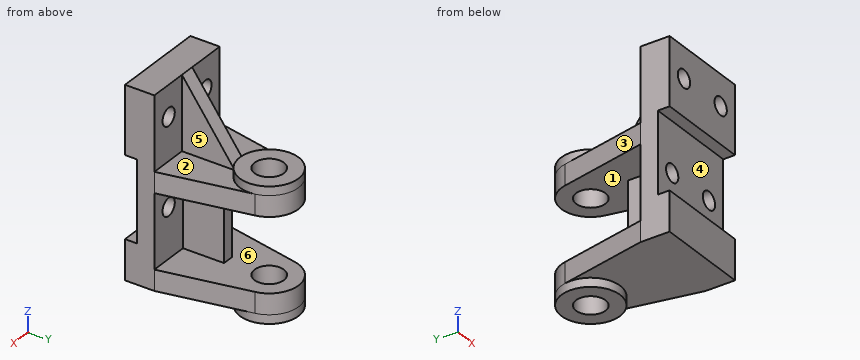
```python
from build123d import *

# Parameters (mm, degrees)
BASE_PLATE_DEPTH           = 32
LUG_UPRIGHT_PROFILE_R      = 10
LUG_UPRIGHT_DEPTH          = 14
LUG_START                  = 6
SKETCH2_3_R                = 20
SKETCH2_3_R_2              = 10
LUG_HUB_BOSS_DEPTH         = 6
BACK_WEB_PROFILE_W         = 8
BACK_WEB_PROFILE_H         = 50
BACK_WEB_DEPTH             = 28
STIFFENING_RIB_REACH       = 165.169
STIFFENING_RIB_PATH_WALL_W = 389.948936072
STIFFENING_RIB_PATH_WALL_H = 10
MOUNTING_HOLES_PROFILE_R   = 6
MOUNTING_HOLES_DEPTH       = 153.262930485


with BuildPart() as part:
    # Base Plate Profile → Base Plate (new, symmetric)
    with BuildSketch(Plane(origin=(0, 0, 0), x_dir=(0, 0, -1), z_dir=(1, 0, 0))):
        Polygon((-82, 0), (-128, 0), (-128, 20), (0, 20), (0, 0), (-27, 0), (-27, 8), (-82, 8), align=None)
    extrude(amount=BASE_PLATE_DEPTH, both=True)

    # Lug Upright Profile → Lug Upright (add)
    with BuildSketch(Plane(origin=(0, 0, 0), x_dir=(-1, 0, 0), z_dir=(0, 0, -1))):
        with BuildLine():
            Line((-19.585841233, 80.049052133), (-32, 20))
            Line((-32, 20), (32, 20))
            Line((32, 20), (19.585841233, 80.049052133))
            ThreePointArc((19.585841233, 80.049052133), (0, 96), (-19.585841233, 80.049052133))
        make_face()
        with Locations((0, 76)):
            Circle(LUG_UPRIGHT_PROFILE_R, mode=Mode.SUBTRACT)
    lug_upright = extrude(amount=-LUG_UPRIGHT_DEPTH)

    # Sketch2_3 → Lug Hub Boss (add)
    with BuildSketch(Plane(origin=(0, 0, 0), x_dir=(-1, 0, 0), z_dir=(0, 0, -1)).offset(LUG_START)):
        with Locations((0, 76)):
            Circle(SKETCH2_3_R)
        with Locations((0, 76)):
            Circle(SKETCH2_3_R_2, mode=Mode.SUBTRACT)
    lug_hub_boss = extrude(amount=-LUG_HUB_BOSS_DEPTH)

    # Lug Mirror: Lug Upright, Lug Hub Boss across plane
    add(lug_upright.mirror(Plane.XY.offset(39)))
    add(lug_hub_boss.mirror(Plane.XY.offset(39)))

    # Back Web Profile → Back Web (add)
    with BuildSketch(Plane(origin=(0, 20, 0), x_dir=(1, 0, 0), z_dir=(0, 1, 0))):
        with Locations((0, -39)):
            Rectangle(BACK_WEB_PROFILE_W, BACK_WEB_PROFILE_H)
    extrude(amount=BACK_WEB_DEPTH)

    # Stiffening Rib Path wall → Stiffening Rib (add, up to next)
    with BuildSketch(Plane(origin=(0, 38, 103), x_dir=(0, 0.584304725845, -0.811534341451), z_dir=(0, 0.811534341451, 0.584304725845)), mode=Mode.PRIVATE) as stiffening_rib_sk1:
        Rectangle(STIFFENING_RIB_PATH_WALL_W, STIFFENING_RIB_PATH_WALL_H)
    stiffening_rib_tool1 = extrude(stiffening_rib_sk1.sketch, amount=-STIFFENING_RIB_REACH, mode=Mode.PRIVATE) - part.part
    add(stiffening_rib_tool1.solids().sort_by_distance((0, 38, 103))[0])

    # Mounting Holes Profile → Mounting Holes (cut, through all)
    with BuildSketch(Plane(origin=(0, 20, 0), x_dir=(1, 0, 0), z_dir=(0, 1, 0))):
        with Locations(Location((-18, -48, 0), (0, 0, 270))):
            Circle(MOUNTING_HOLES_PROFILE_R)
        with Locations(Location((18, -48, 0), (0, 0, 270))):
            Circle(MOUNTING_HOLES_PROFILE_R)
        with Locations(Location((18, -107, 0), (0, 0, 270))):
            Circle(MOUNTING_HOLES_PROFILE_R)
        with Locations(Location((-18, -107, 0), (0, 0, 270))):
            Circle(MOUNTING_HOLES_PROFILE_R)
    extrude(amount=-MOUNTING_HOLES_DEPTH, mode=Mode.SUBTRACT)


solid = part.part
```
Check sheet for the modelled part. Datum: model origin and axes. Units: mm. Face numbers are marked on the shaded views. A direction names the side the tool comes from. Give positions to 0.01 mm unless a question says otherwise; leave off trailing zeros. Order: outer loops, then holes, each group sorted by start corner. A loop starts at its lowest first (then second) coordinate and runs counter-clockwise, first axis right, second up. Notation, with made-up numbers: M 64.25,23 L 69.25,23 A26 cw 69.25,40 Z; hole C -8.75,-30.75 d9. An arc over 180 degrees is marked long. Answer in a Markdown table with one row per item. Add a question column.
Q1. Sectioned sample at A-A, the plane z = 48. Record the boundary of the cut face in (x, y).
Q2. Release check for a two-part mould opening along Z. For the marked faces 1, 2 and 3 record: released by +Z, released by -Z, zero draft, split by the parting line, or undercut.
Q3. Sectioned sample at C-C, the plane z = 6. Record the boundary of the cut face in (x, y), and give its area (3 significant figures).
Q4. Gauge pin test, flat ends, axial feed: pin 1 Ø4 at (x, y) = (23.5, 37) entering from +Z; pin 2 Ø14 at (y, z) = (27.5, 31.5) entering from +X; pin 3 Ø14 at (x, z) = (18, 48) entering from +Y. Record the tip position at first contact, or that the pin passes through.
Q5. Access from +Z, -Z, +X, -X, +Y, -Y to the whole of each face (thin tool, end or side, straight path). Record for the marked faces 4, 5 and 6.
Q6. Sectioned sample at D-D, the plane x = 18. Record the boundary of the cut face in (y, z), and give its area (3 significant figures).
Q7. Thickness scan on L1, parallel to X at y = 14, z = 107; L2, parallel to Z at x = 26, y = 39; L3, parallel to Y at x = 0, z = 9. Record the ranges inside material, lowest first.
Q8. Sectioned sample at B-B, the plane y = 10. Record the boundary of the cut face in (x, z).
Verdict:
| question | item | result |
|---|---|---|
| 1 | outline | M -32,8 L -24,8 L -24,20 L -32,20 Z; M -12,8 L 12,8 L 12,20 L 4,20 L 4,48 L -4,48 L -4,20 L -12,20 Z; M 24,8 L 32,8 L 32,20 L 24,20 Z |
| 2 | face 1 | undercut |
| 2 | face 2 | released by +Z |
| 2 | face 3 | zero draft |
| 3 | outline | M -32,0 L 32,0 L 32,20 L 19.59,80.05 A20 ccw -19.59,80.05 L -32,20 Z; hole C 0,76 d20 |
| 3 | area | 4,530 mm² |
| 4 | pin 1 | z = 78 |
| 4 | pin 2 | x = 4 |
| 4 | pin 3 | y = 20 |
| 5 | face 4 | +X, -X, -Y |
| 5 | face 5 | +Z, +X |
| 5 | face 6 | +Y |
| 6 | outline | M 0,0 L 67.28,0 L 67.28,-6 L 84.72,-6 L 84.72,14 L 20,14 L 20,42 L 8,42 L 8,27 L 0,27 Z; M 0,82 L 8,82 L 8,54 L 20,54 L 20,64 L 84.72,64 L 84.72,84 L 67.28,84 L 67.28,78 L 20,78 L 20,101 L 0,101 Z; M 0,113 L 20,113 L 20,128 L 0,128 Z |
| 6 | area | 3,760 mm² |
| 7 | L1 | -32 to -24, -12 to 12, 24 to 32 |
| 7 | L2 | 0 to 14, 64 to 78 |
| 7 | L3 | 0 to 66, 86 to 96 |
| 8 | outline | M -32,0 L 32,0 L 32,128 L -32,128 Z; hole C -18,48 d12; hole C -18,107 d12; hole C 18,48 d12; hole C 18,107 d12 |
